Here's how the part is built. I have some questions about the finished solid (model axes, mm). Face numbers are marked on the shaded views. A direction names the side the tool comes from. Round coordinates to 2 decimals unless told otherwise and drop trailing zeros. Order: outer loops, then holes, each group sorted by start corner. A loop starts at its lowest first (then second) coordinate and runs counter-clockwise, first axis right, second up. Notation, with made-up numbers: M 50.5,5 L 101.5,5 A7 cw 101.5,14 Z; hole C 51,-35.75 d10. An arc over 180 degrees is marked long. Write item = value, one per line. Start each with the question number.
Item 1: I want a section at B-B, the plane y = 14.5. List the corners of the cut face in (x, z) for me, plus the area to 3 significant figures.
Item 2: I want a section at C-C, the plane z = 7.25. List the corners of the cut face in (x, y) for me, plus the area to 3 significant figures.
Item 3: We'd pull the mould along Z, two halves only. Please class the marked faces 1, 2 and 3: pulls with the +Z half, pulls with the -Z half, needs draft (parallel to the pull), parting line crosses it, or undercut.
Item 4: For the marked faces 4, 5 and 6, which set-ups out of +Z, -Z, +X, -X, +Y, -Y let a thin tool reach every point of the face, with its end or its side?
Item 5: I want a section at D-D, the plane x = 5.5. List the corners of the cut face in (y, z) for me, plus the area to 3 significant figures.
Item 6: I want a section at A-A, the plane x = 2.75. List the corners of the cut face in (y, z) for me, plus the area to 3 significant figures.
Item 7: Please list where these lines run through material, in increasing order: L1, parallel to Z at x = 4.4, y = 15; L2, parallel to Y at x = 3.5, z = 4; L3, parallel to X at y = 3.75, z = -0.25.
Item 8: I'm going to push flat-ended pins straight in: P1, Ø9, axis at y = 8.5, z = 4, coming from the +X side; P2, Ø0.8, axis at x = 5, z = 0.5, coming from the -Y side; P3, Ø0.8, axis at y = 20.5, z = -2.5, coming from the +X side; P4, Ø1.8, axis at y = 15, z = -4, coming from the +X side. Where does each tip first touch, or does it pass through?
```python
from build123d import *

# Parameters (mm, degrees)
EXTRUDE_1_DEPTH     = 9
SKETCH_2_W          = 8
SKETCH_2_H          = 15
CUT_EXTRUDE_1_DEPTH = 1.5
CUT_EXTRUDE_2_REACH = 34.469
SKETCH_3_R          = 1.5
SKETCH_4_W          = 18
SKETCH_4_H          = 1.5
CUT_EXTRUDE_3_DEPTH = 1.5
CHAMFER_1_SIZE      = 8


with BuildPart() as part:
    # 草图1 → 凸台-拉伸1 (new, symmetric)
    with BuildSketch(Plane.XY):
        Polygon((0, 0), (0, 29), (17.5, 29), (17.5, 19), (6, 19), (6, 0), align=None)
    extrude(amount=EXTRUDE_1_DEPTH, both=True)

    # 草图2 → 切除-拉伸1 (cut)
    with BuildSketch(Plane(origin=(6, 0, 0), x_dir=(0, 0, -1), z_dir=(1, 0, 0))):
        with Locations((0, 7.5)):
            Rectangle(SKETCH_2_W, SKETCH_2_H)
    extrude(amount=-CUT_EXTRUDE_1_DEPTH, mode=Mode.SUBTRACT)

    # 草图3 → 切除-拉伸2 (cut, up to next)
    with BuildSketch(Plane(origin=(6, 0, 0), x_dir=(0, 0, -1), z_dir=(1, 0, 0)), mode=Mode.PRIVATE) as cut_extrude_2_sk1:
        with Locations(Location((4, 15, 0), (0, 0, 180))):
            Circle(SKETCH_3_R)
    cut_extrude_2_tool1 = extrude(cut_extrude_2_sk1.sketch, amount=-CUT_EXTRUDE_2_REACH, mode=Mode.PRIVATE) & part.part
    # 草图3 → 切除-拉伸2 (cut, up to next)
    with BuildSketch(Plane(origin=(6, 0, 0), x_dir=(0, 0, -1), z_dir=(1, 0, 0)), mode=Mode.PRIVATE) as cut_extrude_2_sk2:
        with Locations((-4, 15)):
            Circle(SKETCH_3_R)
    cut_extrude_2_tool2 = extrude(cut_extrude_2_sk2.sketch, amount=-CUT_EXTRUDE_2_REACH, mode=Mode.PRIVATE) & part.part
    add(cut_extrude_2_tool1.solids().sort_by_distance((6, 15, -4))[0], mode=Mode.SUBTRACT)
    add(cut_extrude_2_tool2.solids().sort_by_distance((6, 15, 4))[0], mode=Mode.SUBTRACT)

    # 草图4 → 切除-拉伸3 (cut)
    with BuildSketch(Plane(origin=(17.5, 0, 0), x_dir=(0, 0, -1), z_dir=(1, 0, 0))):
        with Locations((0, 26.75)):
            Rectangle(SKETCH_4_W, SKETCH_4_H)
        with Locations((0, 23.75)):
            Rectangle(SKETCH_4_W, SKETCH_4_H)
        with Locations((0, 20.75)):
            Rectangle(SKETCH_4_W, SKETCH_4_H)
    extrude(amount=-CUT_EXTRUDE_3_DEPTH, mode=Mode.SUBTRACT)

    # 倒角1
    chamfer_1_edges = [part.edges().sort_by_distance(p)[0] for p in [
        (0, 29, 0),
    ]]
    chamfer(chamfer_1_edges, length=CHAMFER_1_SIZE)


solid = part.part
```
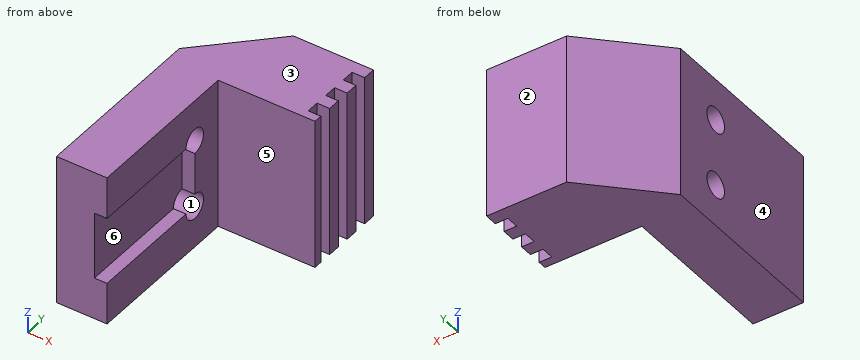
Filled in:
q1.outline = M 0,-9 L 6,-9 L 6,-5.41 L 0,-5.41 Z; M 0,-2.59 L 4.5,-2.59 L 4.5,2.59 L 0,2.59 Z; M 0,5.41 L 6,5.41 L 6,9 L 0,9 Z
q1.area = 66.3 mm^2
q2.outline = M 0,0 L 6,0 L 6,19 L 17.5,19 L 17.5,20 L 16,20 L 16,21.5 L 17.5,21.5 L 17.5,23 L 16,23 L 16,24.5 L 17.5,24.5 L 17.5,26 L 16,26 L 16,27.5 L 17.5,27.5 L 17.5,29 L 8,29 L 0,21 Z
q2.area = 250 mm^2
q3.face_1 = undercut
q3.face_2 = needs draft
q3.face_3 = pulls with the +Z half
q4.face_4 = +Z, -Z, -X, +Y, -Y
q4.face_5 = +Z, -Z, +X, -Y
q4.face_6 = +X, -Y
q5.outline = M 0,-9 L 26.5,-9 L 26.5,9 L 0,9 L 0,4 L 13.5,4 A1.5 cw long 15,2.5 L 15,-2.5 A1.5 cw long 13.5,-4 L 0,-4 Z
q5.area = 346 mm^2
q6.outline = M 0,-9 L 23.75,-9 L 23.75,9 L 0,9 Z; hole C 15,-4 d3; hole C 15,4 d3
q6.area = 413 mm^2
q7.L1 = -9 to -5.5, -2.5 to 2.5, 5.5 to 9
q7.L2 = 0 to 13.5, 16.5 to 24.5
q7.L3 = 0 to 4.5
q8.P1 = 6
q8.P2 = 15
q8.P3 = 16
q8.P4 = through
